Read the model definition and answer for the solid it produces. Units are mm, in the model's axes. Give positions to 0.01 mm unless a question says otherwise; leave off trailing zeros. Order: outer loops, then holes, each group sorted by start corner. A loop starts at its lowest first (then second) coordinate and runs counter-clockwise, first axis right, second up. Notation, with made-up numbers: (-7, 51.25) - (7, 51.25) arc R23 cw to (7, 85.25) - close; hole circle Ø8 at (80, -22). An arc over 180 degrees is marked (long way). Return JSON: item names as keys, results as strings.
```python
from build123d import *

# Parameters (mm, degrees)
BASE_EXTRUDE_DEPTH = 5
SKETCH2_R          = 5
CUT_EXTRUDE1_DEPTH = 51.069951068


with BuildPart() as part:
    # Sketch1 → Base-Extrude (new body)
    with BuildSketch(Plane.XY):
        with BuildLine():
            Line((0, 9), (40, 9))
            ThreePointArc((40, 9), (49, 0), (40, -9))
            Line((40, -9), (0, -9))
            ThreePointArc((0, -9), (-9, 0), (0, 9))
        make_face()
    extrude(amount=BASE_EXTRUDE_DEPTH)

    # Sketch2 → Cut-Extrude1 (cut, through all)
    with BuildSketch(Plane.XY.offset(5)):
        Circle(SKETCH2_R)
        with Locations((40, 0)):
            Circle(SKETCH2_R)
    extrude(amount=-CUT_EXTRUDE1_DEPTH, mode=Mode.SUBTRACT)


solid = part.part
```
Q1. Consider L1, parallel to X at y = 0.25, z = 4.6; L2, parallel to Y at x = 40, z = 1.95; L3, parallel to X at y = -3.5, z = 0.3. Determine where each line is inside the solid, lowest interval first.
Values:
{"L1": "x = -9 to -4.99, 4.99 to 35.01, 44.99 to 49", "L2": "y = -9 to -5, 5 to 9", "L3": "x = -8.29 to -3.57, 3.57 to 36.43, 43.57 to 48.29"}
Q2. A cutting plane is placed at B-B (x = -2). Write down the section's boundary in (y, z).
Values:
{"outline": "(-8.77, 0) - (-4.58, 0) - (-4.58, 5) - (-8.77, 5) - close; (4.58, 0) - (8.77, 0) - (8.77, 5) - (4.58, 5) - close"}
Q3. A cutting plane is placed at A-A (y = 0). Write down the section's boundary in (x, z).
Values:
{"outline": "(-9, 0) - (-5, 0) - (-5, 5) - (-9, 5) - close; (5, 0) - (35, 0) - (35, 5) - (5, 5) - close; (45, 0) - (49, 0) - (49, 5) - (45, 5) - close"}
Q4. A cutting plane is placed at C-C (z = 3.4). Write down the section's boundary in (x, y).
Values:
{"outline": "(0, -9) - (40, -9) arc R9 ccw to (40, 9) - (0, 9) arc R9 ccw to start; hole circle Ø10 at (0, 0); hole circle Ø10 at (40, 0)"}
Q5. Given pin 1 (1.5 mm diameter, centred on y = -7, z = 1.5, fed in from -X); pin 2 (1.5 mm diameter, centred on x = -2, z = 2.5, fed in from +Y); pin 3 (6 mm diameter, centred on x = 0, y = 0, fed in from +Z), each flat-ended and moving along its own axis, determine where each tip first touches the part or whether it passes through.
Values:
{"pin 1": "stops at x = -6.48", "pin 2": "stops at y = 8.91", "pin 3": "passes through"}
Q6. A cutting plane is placed at D-D (x = 37.5). Write down the section's boundary in (y, z), and give its area (3 significant figures).
Values:
{"outline": "(-9, 0) - (-4.33, 0) - (-4.33, 5) - (-9, 5) - close; (4.33, 0) - (9, 0) - (9, 5) - (4.33, 5) - close", "area": "46.7 mm²"}
Q7. Determine the mould class of faces 1 (the cylindrical face through (49, 0, 2)), 2 (the cylindrical face through (35, 0, 3)), 3 (the flat face through (20, 0, 5)) for opening direction X: released by +X, released by -X, zero draft, split by the parting line, or undercut.
Values:
{"face 1": "released by +X", "face 2": "undercut", "face 3": "zero draft"}
